The model under review builds one solid part; all positions refer to its coordinate system, in mm. A direction names the side the tool comes from. Give positions to 0.01 mm unless a question says otherwise; leave off trailing zeros. Loops run counter-clockwise (first coordinate to the right, second up) from the corner with the lowest first, then second, coordinate; pieces in that order, holes last. Notation, with made-up numbers: M 39,-28.5 L 80,-28.5 A29 cw 80,-7.5 Z; hole C 42.5,65.5 d10. An arc over 180 degrees is marked long. One line per item, written item: value. Start each with the question number.
Q1. Mouldability with a two-part tool opening along X and no side actions: class faces 1 (the face through (-5, 0, -42)), 2 (the face through (11.945, -22.033, -20.803)), 3 (the face through (11.625, 21.977, -20.803)), 4 (the face through (0, 0, -56.5)) as released by +X, released by -X, zero draft, split by the parting line, or undercut.
Q2. We need section C-C on z = -45.5. Write out the cut boundary in (x, y), plus the area to 3 significant figures.
Q3. We need section A-A on x = 0. Write out the cut boundary in (y, z).
Q4. For pin 1 (4 mm diameter, centred on y = 4, z = -13.5, fed in from -X); pin 2 (4 mm diameter, centred on x = 12, y = -20.78, fed in from -Z); pin 3 (2 mm diameter, centred on x = 7, y = 17.5, fed in from -Z), all flat-tipped, find the tip position at first contact; note any pin that passes through.
Q5. To check wall thickness, follow line 1 along Z through (x, y) = (10.5, 18); line 2 along X through (y, z) = (-15.5, -10); line 3 along Z through (x, y) = (9, -2). State the ranges of each line that lie inside material, in increasing order. Write a range as from..to.
Q6. We need section B-B on z = -6. Write out the cut boundary in (x, y), plus the area to 3 significant figures.
Q7. For faces 5 (the face through (-13.3, -12.5, -24.5)), 6 (the face through (13.38, -25.73, -1.18)), list the 3-axis set-ups (+Z, -Z, +X, -X, +Y, -Y) from which the entire face can be reached by the end or side of a thin tool; tool diameter is ignored.
```python
from build123d import *

# Parameters (mm, degrees)
SKETCH_1_R               = 29
EXTRUDE_1_DEPTH          = 24.5
FILLET_1_R               = 3
SKETCH_2_R               = 5
EXTRUDE_2_DEPTH          = 32
PATTERN_CIRCULAR_1_COUNT = 3
SKETCH_5_R               = 18
EXTRUDE_3_DEPTH          = 2.5


with BuildPart() as part:
    # 草图1 → 凸台-拉伸1 (new, symmetric)
    with BuildSketch(Plane.XY):
        Circle(SKETCH_1_R)
    extrude(amount=EXTRUDE_1_DEPTH, both=True)

    # 圆角1
    fillet_1_edges = [part.edges().sort_by_distance(p)[0] for p in [
        (-29, 0, 24.5),
    ]]
    fillet(fillet_1_edges, radius=FILLET_1_R)

    # 草图2 → 凸台-拉伸2 (add)
    with BuildSketch(Plane(origin=(0, 0, -24.5), x_dir=(-1, 0, 0), z_dir=(0, 0, -1))):
        with Locations(Location((0, 0, 0), (0, 0, 180))):
            Circle(SKETCH_2_R)
    extrude(amount=EXTRUDE_2_DEPTH)

    # 草图3 → M3 螺纹孔1 (revolve, cut)
    with BuildSketch(Plane(origin=(-24, 0, -24.5), x_dir=(0, 1, 0), z_dir=(1, 0, 0))):
        Polygon((0, 0), (0, 8.251075774), (1.25, 7.5), (1.25, 0), align=None)
    hole_wizard_m3_1 = revolve(axis=Axis((-24, 0, -30.85), (0, 0, 1)), mode=Mode.SUBTRACT)

    # 阵列(圆周)1: M3 螺纹孔1 ×3 about axis
    pattern_circular_1_axis = Axis((0, 0, 0), (0, 0, 1))
    for i in range(1, PATTERN_CIRCULAR_1_COUNT):
        add(hole_wizard_m3_1.rotate(pattern_circular_1_axis, i * 360 / PATTERN_CIRCULAR_1_COUNT), mode=Mode.SUBTRACT)

    # 草图5 → 凸台-拉伸3 (add)
    with BuildSketch(Plane(origin=(0, 0, -24.5), x_dir=(-1, 0, 0), z_dir=(0, 0, -1))):
        with Locations(Location((0, 0, 0), (0, 0, 180))):
            Circle(SKETCH_5_R)
    extrude(amount=EXTRUDE_3_DEPTH)


solid = part.part
```
Solved:
1. face 1: split by the parting line
1. face 2: undercut
1. face 3: undercut
1. face 4: zero draft
2. outline: C 0,0 d10
2. area: 78.5 mm2
3. outline: M -29,-24.5 L -18,-24.5 L -18,-27 L -5,-27 L -5,-56.5 L 5,-56.5 L 5,-27 L 18,-27 L 18,-24.5 L 29,-24.5 L 29,21.5 A3 ccw 26,24.5 L -26,24.5 A3 ccw -29,21.5 Z
4. pin 1: x = -28.93
4. pin 2: z = -24.5
4. pin 3: z = -27
5. line 1: -24.5..24.5
5. line 2: -24.51..24.51
5. line 3: -27..24.5
6. outline: C 0,0 d58
6. area: 2,640 mm2
7. face 5: -Z
7. face 6: +Z, -Z
